from build123d import *

# Parameters (mm, degrees)
SKETCH1_W           = 1000
SKETCH1_H           = 570
BOSS_EXTRUDE1_DEPTH = 35
M20_TAPPED_HOLE1_D  = 17.5
CUT_EXTRUDE2_DEPTH  = 1152.575008412


with BuildPart() as part:
    # Sketch1 → Boss-Extrude1 (new body)
    with BuildSketch(Plane.XY):
        with Locations((500, 285)):
            Rectangle(SKETCH1_W, SKETCH1_H)
    extrude(amount=BOSS_EXTRUDE1_DEPTH)

    # M20 Tapped Hole1 (through all)
    with Locations(Plane(origin=(30, 285, 35), x_dir=(1, 0, 0), z_dir=(0, 0, 1))):
        with Locations((0, 0)):
            Hole(M20_TAPPED_HOLE1_D / 2)

    # Sketch4 → Cut-Extrude2 (cut, through all)
    with BuildSketch(Plane.XZ):
        Polygon((500, 35), (1000, 35), (1000, -365), align=None)
    extrude(amount=-CUT_EXTRUDE2_DEPTH, mode=Mode.SUBTRACT)


solid = part.part
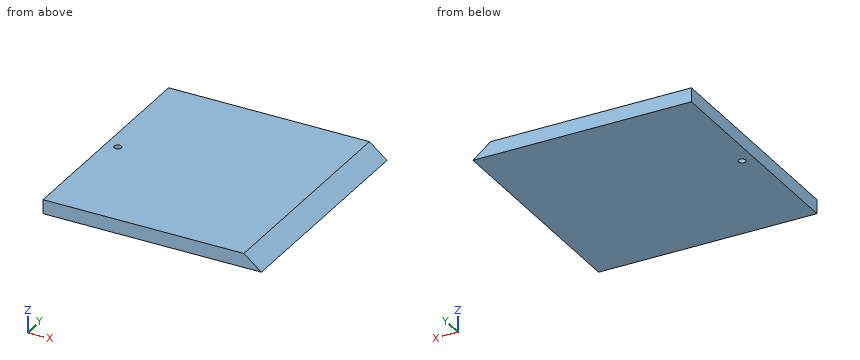
The model under review builds one solid part; all positions refer to its coordinate system, in mm. Round coordinates to 2 decimals unless told otherwise and drop trailing zeros. Write each loop counter-clockwise with the first axis right and the second up, starting at its lowest first coordinate (ties: lowest second). Pieces come first, ordered by that corner, then holes. Notation, with made-up numbers: (-5, 42.25) -> (50, 42.25) arc R23 ccw to (50, 54.25) -> close; hole circle Ø2 at (27, 56). An arc over 180 degrees is marked (long way). Answer as a JSON object with one key per item and string values.
1. We need section C-C on z = 23. State the section outline as (x, y) points.
Results found:
{"outline": "(0, 0) -> (515, 0) -> (515, 570) -> (0, 570) -> close; hole circle Ø17.5 at (30, 285)"}
2. Clearance check with a flat-ended pin moving along its axis: pin 1 (1 mm diameter, centred on y = 328.5, z = 26, fed in from +X) (3 decimals). State where the tip first meets the part, or that it passes through.
Results found:
{"pin 1": "stops at x = 511.875"}
3. We need section D-D on y = 436. State the section outline as (x, z) points.
Results found:
{"outline": "(0, 0) -> (543.75, 0) -> (500, 35) -> (0, 35) -> close"}
4. We need section A-A on y = 285. State the section outline as (x, z) points.
Results found:
{"outline": "(0, 0) -> (21.25, 0) -> (21.25, 35) -> (0, 35) -> close; (38.75, 0) -> (543.75, 0) -> (500, 35) -> (38.75, 35) -> close"}
5. To check wall thickness, follow line 1 along Y through (x, z) = (30, 23.5); line 2 along X through (y, z) = (85.5, 31); line 3 along X through (y, z) = (314, 8). State the ranges of each line that lie inside material, in increasing order.
Results found:
{"line 1": "y = 0 to 276.25, 293.75 to 570", "line 2": "x = 0 to 505", "line 3": "x = 0 to 533.75"}
6. We need section B-B on x = 30. State the section outline as (y, z) points.
Results found:
{"outline": "(0, 0) -> (276.25, 0) -> (276.25, 35) -> (0, 35) -> close; (293.75, 0) -> (570, 0) -> (570, 35) -> (293.75, 35) -> close"}
